from build123d import *

# Parameters (mm, degrees)
BOSS_EXTRUDE1_DEPTH         = 22
BOSS_EXTRUDE2_DEPTH         = 5
BOSS_EXTRUDE3_DEPTH         = 5
SKETCH_4_3_2_R              = 5
BOSS_EXTRUDE4_DEPTH         = 11
M8_TAPPED_HOLE1_D           = 6.8
M8_TAPPED_HOLE1_DEPTH       = 19.957073895
M8_TAPPED_HOLE1_CSINK_D     = 8.05
M8_TAPPED_HOLE1_CSINK_ANGLE = 90
M8_TAPPED_HOLE1_TIP         = 2.042926105


with BuildPart() as part:
    # Sketch1 → Boss-Extrude1 (new body)
    with BuildSketch(Plane.XY):
        with BuildLine():
            Line((-20, -13.5), (20, -13.5))
            ThreePointArc((20, -13.5), (23.535533906, -12.035533906), (25, -8.5))
            Line((25, -8.5), (25, 8.5))
            ThreePointArc((25, 8.5), (23.535533906, 12.035533906), (20, 13.5))
            Line((20, 13.5), (-20, 13.5))
            ThreePointArc((-20, 13.5), (-23.535533906, 12.035533906), (-25, 8.5))
            Line((-25, 8.5), (-25, -8.5))
            ThreePointArc((-25, -8.5), (-23.535533906, -12.035533906), (-20, -13.5))
        make_face()
    extrude(amount=BOSS_EXTRUDE1_DEPTH)

    # Sketch2 → Boss-Extrude2 (add)
    with BuildSketch(Plane.XY.offset(22)):
        with BuildLine():
            Line((-12, -11), (12, -11))
            ThreePointArc((12, -11), (17.656854249, -8.656854249), (20, -3))
            Line((20, -3), (20, 3))
            ThreePointArc((20, 3), (17.656854249, 8.656854249), (12, 11))
            Line((12, 11), (-12, 11))
            ThreePointArc((-12, 11), (-17.656854249, 8.656854249), (-20, 3))
            Line((-20, 3), (-20, -3))
            ThreePointArc((-20, -3), (-17.656854249, -8.656854249), (-12, -11))
        make_face()
    extrude(amount=BOSS_EXTRUDE2_DEPTH)

    # Sketch 4_3 → Boss-Extrude3 (add, symmetric)
    with BuildSketch(Plane(origin=(0, 0, 0), x_dir=(1, 0, 0), z_dir=(0, 1, 0))):
        with BuildLine():
            ThreePointArc((31.338769383, 87.11590511), (23.260937212, 76.86922385), (10.8, 73))
            Line((10.8, 73), (10.8, 0))
            Line((10.8, 0), (25, 0))
            ThreePointArc((25, 0), (18.831156894, 4.245196236), (17.339679571, 11.583575604))
            Line((17.339679571, 11.583575604), (31.338769383, 87.11590511))
        make_face()
        with BuildLine():
            ThreePointArc((10.8, 73), (-1.660937212, 76.86922385), (-9.738769383, 87.11590511))
            Line((-9.738769383, 87.11590511), (4.260320429, 11.583575604))
            ThreePointArc((4.260320429, 11.583575604), (2.768843106, 4.245196236), (-3.4, 0))
            Line((-3.4, 0), (10.8, 0))
            Line((10.8, 0), (10.8, 73))
        make_face()
    extrude(amount=BOSS_EXTRUDE3_DEPTH, both=True)

    # Sketch 4_3 2 → Boss-Extrude4 (add, symmetric)
    with BuildSketch(Plane(origin=(0, 0, 0), x_dir=(1, 0, 0), z_dir=(0, 1, 0))):
        with BuildLine():
            ThreePointArc((32.8, 95), (10.8, 117), (-11.2, 95))
            Line((-11.2, 95), (-9.738769383, 87.11590511))
            ThreePointArc((-9.738769383, 87.11590511), (10.8, 73), (31.338769383, 87.11590511))
            Line((31.338769383, 87.11590511), (32.8, 95))
        make_face()
        with Locations(Location((10.8, 95, 0), (0, 0, 270))):
            Circle(SKETCH_4_3_2_R, mode=Mode.SUBTRACT)
    extrude(amount=BOSS_EXTRUDE4_DEPTH, both=True)

    # M8 Tapped Hole1
    with Locations(Plane(origin=(-10, 0, 27), x_dir=(1, 0, 0), z_dir=(0, 0, 1))):
        with Locations((0, 0), (20, 0)):
            CounterSinkHole(M8_TAPPED_HOLE1_D / 2, M8_TAPPED_HOLE1_CSINK_D / 2, depth=M8_TAPPED_HOLE1_DEPTH, counter_sink_angle=M8_TAPPED_HOLE1_CSINK_ANGLE)
            with Locations((0, 0, -(M8_TAPPED_HOLE1_DEPTH + M8_TAPPED_HOLE1_TIP / 2))):  # 118° drill point
                Cone(0, M8_TAPPED_HOLE1_D / 2, M8_TAPPED_HOLE1_TIP, mode=Mode.SUBTRACT)


solid = part.part
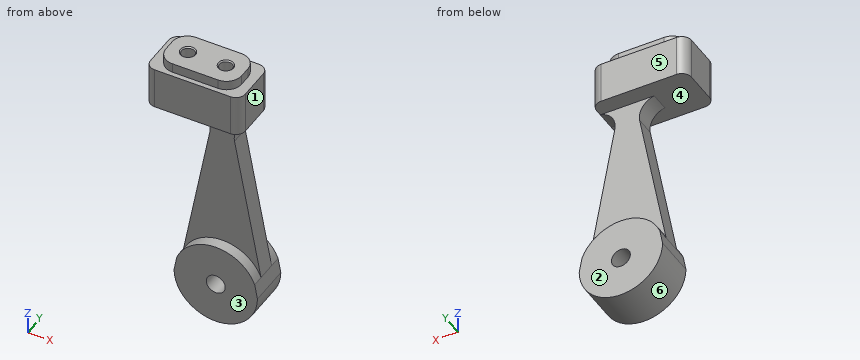
Check sheet for the modelled part. Datum: model origin and axes. Units: mm. Face numbers are marked on the shaded views. A direction names the side the tool comes from. Coordinates: 2 decimals unless noted, no trailing zeros. Write each loop counter-clockwise with the first axis right and the second up, starting at its lowest first coordinate (ties: lowest second). Pieces come first, ordered by that corner, then holes. Notation, with made-up numbers: M 40,26.25 L 93,26.25 A11 ccw 93,43.25 Z; hole C -21,4 d2. An arc over 180 degrees is marked long. Answer as CSV lines item,"result".
Q1. Set-up check for the marked faces 1, 2 and 3: record each of +Z, -Z, +X, -X, +Y, -Y from which the full face is reachable in a straight line by a thin tool's end or side.
Check result:
face 1,"+Z, +X, +Y, -Y"
face 2,"-Z, +X, -X, +Y"
face 3,"-Z, +X, -X, -Y"
Q2. Material ranges on probe 1 along X at (y, z) = (0, 14.5); probe 2 along Y at (x, z) = (10, 11); probe 3 along X at (y, z) = (0.75, -95), recorded low to high. Write a range as from..to.
Check result:
probe 1,"-25..-13.4, -6.6..6.6, 13.4..25"
probe 2,"-13.5..-3.4, 3.4..13.5"
probe 3,"-11.2..5.8, 15.8..32.8"
Q3. Cross-section at A-A (z = -80.5). Record the boundary of the cut face in (x, y), then the cut area to 3 significant figures.
Check result:
outline,"M -8.51,-5 L -5.75,-5 L -5.75,-11 L 27.35,-11 L 27.35,-5 L 30.11,-5 L 30.11,5 L 27.35,5 L 27.35,11 L -5.75,11 L -5.75,5 L -8.51,5 Z"
area,"783 mm^2"
Q4. Cross-section at C-C (z = -38.5). Record the boundary of the cut face in (x, y), then the cut area to 3 significant figures.
Check result:
outline,"M -0.73,-5 L 22.33,-5 L 22.33,5 L -0.73,5 Z"
area,"231 mm^2"
Q5. Go/stop test with flat-tipped pins: pin 1 (2.5 mm diameter, centred on y = -1, z = 25, fed in from -X); pin 2 (1.5 mm diameter, centred on x = 18.5, z = -29.5, fed in from +Y); pin 3 (5 mm diameter, centred on y = -1.5, z = -11, fed in from +X); pin 4 (8 mm diameter, centred on x = 10.8, z = -95, fed in from +Y). Record where each tip stops, or that it passes through.
Check result:
pin 1,"x = -20"
pin 2,"y = 5"
pin 3,"x = 17.69"
pin 4,"through"
Q6. Cross-section at B-B (x = 22.5). Record the boundary of the cut face in (y, z).
Check result:
outline,"M -12.83,0 L -5,0 L -5,-0.92 L 5,-0.92 L 5,0 L 12.83,0 L 12.83,22 L -12.83,22 Z; M -11,-113.63 L 11,-113.63 L 11,-76.37 L 5,-76.37 L 5,-39.43 L -5,-39.43 L -5,-76.37 L -11,-76.37 Z"
Q7. Mould release check, pull along Z, two halves, no side actions. Record for the marked faces 4, 5 and 6: released by +Z, released by -Z, zero draft, split by the parting line, or undercut.
Check result:
face 4,"undercut"
face 5,"zero draft"
face 6,"released by -Z"
